from build123d import *

# Parameters (mm, degrees)
BASE_FLANGE_DEPTH             = 10
SLOT_BOSS_DEPTH               = 22
SLOT_POCKET_DEPTH             = 10
SLOT_THROUGH_CUT_SKETCH_R     = 5
SLOT_THROUGH_CUT_DEPTH        = 53
COUNTERBORES_SKETCH_R         = 6.5
COUNTERBORES_6X_DEPTH_2_DEPTH = 2
MOUNTING_HOLES_SKETCH_R       = 3
MOUNTING_HOLES_6X_DEPTH       = 40


with BuildPart() as part:
    # Base Flange Sketch → Base Flange (new body)
    with BuildSketch(Plane(origin=(0, 0, 0), x_dir=(1, 0, 0), z_dir=(0, 1, 0))):
        with BuildLine():
            Line((-22, -40), (22, -40))
            ThreePointArc((22, -40), (62, 0), (22, 40))
            Line((22, 40), (-22, 40))
            ThreePointArc((-22, 40), (-62, 0), (-22, -40))
        make_face()
    extrude(amount=BASE_FLANGE_DEPTH)

    # Slot Boss Sketch → Slot Boss (add)
    with BuildSketch(Plane(origin=(0, 10, 0), x_dir=(1, 0, 0), z_dir=(0, 1, 0))):
        with BuildLine():
            Line((-22, 16), (22, 16))
            ThreePointArc((22, 16), (38, 0), (22, -16))
            Line((22, -16), (-22, -16))
            ThreePointArc((-22, -16), (-38, 0), (-22, 16))
        make_face()
    extrude(amount=SLOT_BOSS_DEPTH)

    # Slot Pocket Sketch → Slot Pocket (cut)
    with BuildSketch(Plane(origin=(0, 32, 0), x_dir=(1, 0, 0), z_dir=(0, 1, 0))):
        with BuildLine():
            Line((-22, 10), (22, 10))
            ThreePointArc((22, 10), (32, 0), (22, -10))
            Line((22, -10), (-22, -10))
            ThreePointArc((-22, -10), (-32, 0), (-22, 10))
        make_face()
    extrude(amount=-SLOT_POCKET_DEPTH, mode=Mode.SUBTRACT)

    # Slot Through Cut Sketch → Slot Through Cut (cut)
    with BuildSketch(Plane(origin=(0, 22, 0), x_dir=(1, 0, 0), z_dir=(0, 1, 0))):
        with Locations(Location((22, 0, 0), (0, 0, 270))):
            Circle(SLOT_THROUGH_CUT_SKETCH_R)
        with Locations(Location((-22, 0, 0), (0, 0, 270))):
            Circle(SLOT_THROUGH_CUT_SKETCH_R)
    extrude(amount=-SLOT_THROUGH_CUT_DEPTH, mode=Mode.SUBTRACT)

    # Counterbores Sketch → Counterbores 6x Depth 2 (cut)
    with BuildSketch(Plane(origin=(0, 10, 0), x_dir=(1, 0, 0), z_dir=(0, 1, 0))):
        with Locations(Location((48, 0, 0), (0, 0, 270))):
            Circle(COUNTERBORES_SKETCH_R)
        with Locations(Location((22, 26, 0), (0, 0, 270))):
            Circle(COUNTERBORES_SKETCH_R)
        with Locations(Location((-22, 26, 0), (0, 0, 270))):
            Circle(COUNTERBORES_SKETCH_R)
        with Locations(Location((-48, 0, 0), (0, 0, 270))):
            Circle(COUNTERBORES_SKETCH_R)
        with Locations(Location((-22, -26, 0), (0, 0, 270))):
            Circle(COUNTERBORES_SKETCH_R)
        with Locations(Location((22, -26, 0), (0, 0, 270))):
            Circle(COUNTERBORES_SKETCH_R)
    extrude(amount=-COUNTERBORES_6X_DEPTH_2_DEPTH, mode=Mode.SUBTRACT)

    # Mounting Holes Sketch → Mounting Holes 6x (cut)
    with BuildSketch(Plane(origin=(0, 8, 0), x_dir=(1, 0, 0), z_dir=(0, 1, 0))):
        with Locations(Location((48, 0, 0), (0, 0, 270))):
            Circle(MOUNTING_HOLES_SKETCH_R)
        with Locations(Location((22, -26, 0), (0, 0, 270))):
            Circle(MOUNTING_HOLES_SKETCH_R)
        with Locations(Location((-22, -26, 0), (0, 0, 270))):
            Circle(MOUNTING_HOLES_SKETCH_R)
        with Locations(Location((-48, 0, 0), (0, 0, 270))):
            Circle(MOUNTING_HOLES_SKETCH_R)
        with Locations(Location((-22, 26, 0), (0, 0, 270))):
            Circle(MOUNTING_HOLES_SKETCH_R)
        with Locations(Location((22, 26, 0), (0, 0, 270))):
            Circle(MOUNTING_HOLES_SKETCH_R)
    extrude(amount=-MOUNTING_HOLES_6X_DEPTH, mode=Mode.SUBTRACT)


solid = part.part
Could you check a few things on this model? Use its own coordinates, in mm. A direction names the side the tool comes from. Give positions to 0.01 mm unless a question says otherwise; leave off trailing zeros. Order: outer loops, then holes, each group sorted by start corner. A loop starts at its lowest first (then second) coordinate and runs counter-clockwise, first axis right, second up. Notation, with made-up numbers: (32, 65) -> (82, 65) arc R12 cw to (82, 86) -> close; hole circle Ø5 at (-9, 59). An arc over 180 degrees is marked (long way). Answer in a Markdown table with one row per item. Add a question column.
Item 1: Imagine slicing it at B-B (y = 3). Count the separate pieces of the cut face and the enclosed holes in it, and give its area (3 significant figures).
Item 2: Please list where these lines run through material, in increasing order: probe 1 along Z at (x, y) = (16.5, 24); probe 2 along X at (y, z) = (8.7, 26); probe 3 along X at (y, z) = (4.75, 0).
Item 3: I'm going to push flat-ended pins straight in: P1, Ø12, axis at y = 12.5, z = 13.5, coming from the -X side; P2, Ø10.5, axis at x = 19, z = 24, coming from the +Y side; P3, Ø11, axis at x = -1.5, y = 22.5, coming from the -Z side; P4, Ø15, axis at x = 48, z = 0, coming from the -Y side. Where does each tip first touch, or does it pass through?
Item 4: Imagine slicing it at A-A (y = 25). List the corners of the cut face in (x, z) for me.
Item 5: Imagine slicing it at C-C (x = 48). List the corners of the cut face in (y, z) for me.
Item 6: For faces 5 (the cylindrical face through (22.286, 9.014, 19.506)), 6 (the cylindrical face through (-38, 21, 0)), 7 (the cylindrical face through (61.99, 4.93, 0.88)), which set-ups out of +Z, -Z, +X, -X, +Y, -Y let a thin tool reach every point of the face, with its end or its side?
Item 7: We'd pull the mould along Z, two halves only. Please class faces 1 (the flat face through (-1, 10, 17)), 2 (the cylindrical face through (-23.8, 4.1, -28.4)), 3 (the flat face through (0, 21, 16)), 4 (the cylindrical face through (38, 21, 0)): pulls with the +Z half, pulls with the -Z half, needs draft (parallel to the pull), parting line crosses it, or undercut.
Item 8: Imagine slicing it at D-D (y = 16). List the corners of the cut face in (x, z) for me.
Result:
| question | item | result |
|---|---|---|
| 1 | separate pieces | 1 |
| 1 | enclosed holes | 8 |
| 1 | area | 8,220 mm2 |
| 2 | probe 1 | -16 to -10, 10 to 16 |
| 2 | probe 2 | -52.4 to -28.5, -15.5 to 15.5, 28.5 to 52.4 |
| 2 | probe 3 | -62 to -51, -45 to -27, -17 to 17, 27 to 45, 51 to 62 |
| 3 | P1 | x = -61.18 |
| 3 | P2 | y = 10 |
| 3 | P3 | z = -16 |
| 3 | P4 | y = 0 |
| 4 | outline | (-22, -16) -> (22, -16) arc R16 ccw to (22, 16) -> (-22, 16) arc R16 ccw to start; hole (-22, -10) -> (22, -10) arc R10 ccw to (22, 10) -> (-22, 10) arc R10 ccw to start |
| 5 | outline | (0, -30.4) -> (10, -30.4) -> (10, -6.5) -> (8, -6.5) -> (8, -3) -> (0, -3) -> close; (0, 3) -> (8, 3) -> (8, 6.5) -> (10, 6.5) -> (10, 30.4) -> (0, 30.4) -> close |
| 6 | face 5 | +Y |
| 6 | face 6 | -X, +Y |
| 6 | face 7 | +X, +Y, -Y |
| 7 | face 1 | needs draft |
| 7 | face 2 | undercut |
| 7 | face 3 | pulls with the +Z half |
| 7 | face 4 | parting line crosses it |
| 8 | outline | (-22, -16) -> (22, -16) arc R16 ccw to (22, 16) -> (-22, 16) arc R16 ccw to start; hole circle Ø10 at (-22, 0); hole circle Ø10 at (22, 0) |
